from build123d import *

# Parameters (mm, degrees)
SKETCH1_W              = 210
SKETCH1_H              = 200
BOSS_EXTRUDE1_DEPTH    = 8
CHAMFER1_SIZE          = 50
M12_TAPPED_HOLE1_D     = 10.2
M12_TAPPED_HOLE1_DEPTH = 29.25
M12_TAPPED_HOLE1_TIP   = 3.064389157
SKETCH5_W              = 180.548294757
SKETCH5_H              = 165.829683772
CUT_EXTRUDE1_DEPTH     = 8
CHAMFER2_SIZE          = 5
FILLET1_R              = 10


with BuildPart() as part:
    # Sketch1 → Boss-Extrude1 (new body)
    with BuildSketch(Plane.XY):
        Rectangle(SKETCH1_W, SKETCH1_H)
    extrude(amount=BOSS_EXTRUDE1_DEPTH)

    # Chamfer1
    chamfer1_edges = [part.edges().sort_by_distance(p)[0] for p in [
        (105, -100, 4),
        (-105, -100, 4),
    ]]
    chamfer(chamfer1_edges, length=CHAMFER1_SIZE)

    # M12 Tapped Hole1
    with Locations(Plane.XY.offset(8)):
        with Locations((-75, 75.01), (-75, -24.99)):
            Hole(M12_TAPPED_HOLE1_D / 2, depth=M12_TAPPED_HOLE1_DEPTH)
            with Locations((0, 0, -(M12_TAPPED_HOLE1_DEPTH + M12_TAPPED_HOLE1_TIP / 2))):  # 118° drill point
                Cone(0, M12_TAPPED_HOLE1_D / 2, M12_TAPPED_HOLE1_TIP, mode=Mode.SUBTRACT)

    # Sketch5 → Cut-Extrude1 (cut)
    with BuildSketch(Plane.XY.offset(8)):
        with Locations((75.274147379, 42.914841886)):
            Rectangle(SKETCH5_W, SKETCH5_H)
    extrude(amount=-CUT_EXTRUDE1_DEPTH, mode=Mode.SUBTRACT)

    # Chamfer2
    chamfer2_edges = [part.edges().sort_by_distance(p)[0] for p in [
        (-15, 100, 4),
    ]]
    chamfer(chamfer2_edges, length=CHAMFER2_SIZE)

    # Fillet1
    fillet1_edges = [part.edges().sort_by_distance(p)[0] for p in [
        (-15, -40, 4),
    ]]
    fillet(fillet1_edges, radius=FILLET1_R)


solid = part.part
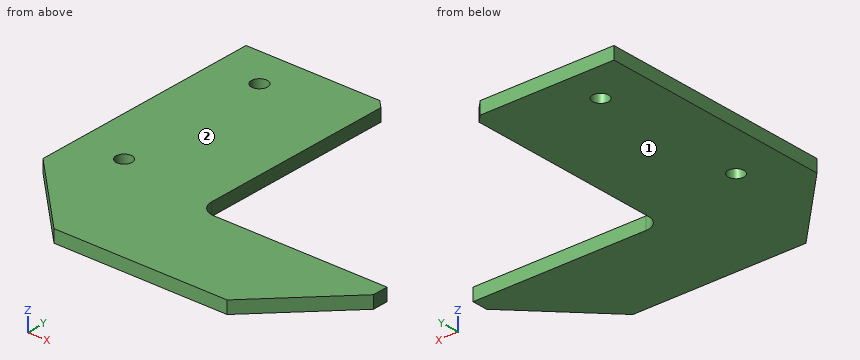
The listing builds one solid part. Answer for the finished solid, in the listing's coordinates (mm). Face numbers are marked on the shaded views. Coordinates: 2 decimals unless noted, no trailing zeros. Order: outer loops, then holes, each group sorted by start corner. A loop starts at its lowest first (then second) coordinate and runs counter-clockwise, first axis right, second up. Notation, with made-up numbers: M 38.5,-23 L 61.5,-23 A27 cw 61.5,7 Z; hole C 67.5,58.25 d5. An arc over 180 degrees is marked long. Use CSV: the item, a comma, the result in double quotes.
Q1. Section D-D (y = 67) is taken. Determine the outline of the cut face in (x, z).
Here are the results:
outline,"M -105,0 L -15,0 L -15,8 L -105,8 Z"
Q2. Given pin 1 Ø11.5 at (x, y) = (-75, -24.99) entering from -Z; pin 2 Ø2.5 at (y, z) = (53, 4.5) entering from +X, each flat-ended and moving along its own axis, determine where each tip first touches the part or whether it passes through.
Here are the results:
pin 1,"z = 0"
pin 2,"x = -15"
Q3. Straight lines are drawn through the part: L1, parallel to Y at x = -75, z = 3.5; L2, parallel to X at y = 75, z = 4; L3, parallel to X at y = 41, z = 6.25. For each, find the intervals that lie inside material, in ascending order.
Here are the results:
L1,"-80 to -30.09, -19.89 to 69.91, 80.11 to 100"
L2,"-105 to -80.1, -69.9 to -15"
L3,"-105 to -15"
Q4. Section C-C (z = 6.5) is taken. Determine the outline of the cut face in (x, y).
Here are the results:
outline,"M -105,-50 L -55,-100 L 55,-100 L 105,-50 L 105,-40 L -5,-40 A10 cw -15,-30 L -15,95 L -20,100 L -105,100 Z; hole C -75,-24.99 d10.2; hole C -75,75.01 d10.2"
Q5. Section A-A (x = -75) is taken. Determine the outline of the cut face in (y, z).
Here are the results:
outline,"M -80,0 L -30.09,0 L -30.09,8 L -80,8 Z; M -19.89,0 L 69.91,0 L 69.91,8 L -19.89,8 Z; M 80.11,0 L 100,0 L 100,8 L 80.11,8 Z"
Q6. Determine the mould class of the marked faces 1 and 2 for opening direction Z: pulls with the +Z half, pulls with the -Z half, needs draft (parallel to the pull), parting line crosses it, or undercut.
Here are the results:
face 1,"pulls with the -Z half"
face 2,"pulls with the +Z half"
Q7. Section B-B (y = -24.99) is taken. Determine the outline of the cut face in (x, z), then the cut area to 3 significant figures.
Here are the results:
outline,"M -105,0 L -80.1,0 L -80.1,8 L -105,8 Z; M -69.9,0 L -15,0 L -15,8 L -69.9,8 Z"
area,"638 mm2"
